Source: CAD feature listing. Evaluate the final solid. Frame: model axes, mm. Round coordinates to 2 decimals unless told otherwise and drop trailing zeros. Order: outer loops, then holes, each group sorted by start corner. A loop starts at its lowest first (then second) coordinate and runs counter-clockwise, first axis right, second up. Notation, with made-up numbers: (45.25, 10.25) -> (50.25, 10.25) arc R12 ccw to (50.25, 21.25) -> close; hole circle Ø4 at (-32.75, 75). An arc over 180 degrees is marked (long way). One line per item, written item: value. Start each with the question number.
1) Section C-C (y = 151.5). Return the cut outline in (x, z).
2) Section A-A (z = 3). Return the cut outline in (x, y), and give its area (4 significant figures).
3) Section B-B (x = -6.5). Return the cut outline in (y, z), and give its area (3 significant figures).
4) Ray query, L1, parallel to X at y = 163, z = 8.5; L2, parallel to X at y = 177, z = 1. Return the intervals inside material, ascending.
```python
from build123d import *

# Parameters (mm, degrees)
SKETCH_1_W          = 60
SKETCH_1_H          = 550
EXTRUDE_1_DEPTH     = 12
CUT_EXTRUDE_1_DEPTH = 12


with BuildPart() as part:
    # 草图1 → 凸台-拉伸1 (new body)
    with BuildSketch(Plane.XY):
        Rectangle(SKETCH_1_W, SKETCH_1_H)
    extrude(amount=EXTRUDE_1_DEPTH)

    # 草图2 → 切除-拉伸1 (cut)
    with BuildSketch(Plane.XY.offset(12)):
        Polygon((-20, 275), (30, 125), (30, 275), align=None)
    extrude(amount=-CUT_EXTRUDE_1_DEPTH, mode=Mode.SUBTRACT)


solid = part.part
```
Findings:
1. outline: (-30, 0) -> (21.17, 0) -> (21.17, 12) -> (-30, 12) -> close
2. outline: (-30, -275) -> (30, -275) -> (30, 125) -> (-20, 275) -> (-30, 275) -> close
2. area: 29,250 mm2
3. outline: (-275, 0) -> (234.5, 0) -> (234.5, 12) -> (-275, 12) -> close
3. area: 6,110 mm2
4. L1: -30 to 17.33
4. L2: -30 to 12.67
